Check sheet for the modelled part. Datum: model origin and axes. Units: mm. A direction names the side the tool comes from. Coordinates: 2 decimals unless noted, no trailing zeros. Loops run counter-clockwise (first coordinate to the right, second up) from the corner with the lowest first, then second, coordinate; pieces in that order, holes last. Notation, with made-up numbers: (-10, 5) - (38, 5) arc R29 cw to (38, 35) - close; hole circle Ø2 at (25.5, 74). An arc over 180 degrees is marked (long way). Use a Markdown table: item, result. Add a question column.
1) Tool access check on faces 1 (the flat face through (-7.922, 11, 7)), 2 (the flat face through (-22.41, -3.21, 14.51)), 3 (the flat face through (23, 1.722, 7)). Record the directions out of +Z, -Z, +X, -X, +Y, -Y that give a thin tool (end or side, any length) a straight path to the whole face; none if there is none.
2) Sectioned sample at A-A, the plane z = 7.5. Enter the section's corners in (x, y).
3) Sectioned sample at B-B, the plane y = -4.5. Enter the section's corners in (x, z).
4) Draft check along X on faces 4 (the flat face through (2, -8.278, 7)), 5 (the flat face through (27.078, -3, 7)), 6 (the cylindrical face through (16.53, -3.35, 8.76)). Enter one of: pulls with the +X half, pulls with the -X half, needs draft (parallel to the pull), parting line crosses it, or undercut.
5) Go/stop test with flat-tipped pins: P1, Ø1.5, axis at y = 4, z = 12, coming from the +X side; P2, Ø1, axis at x = -6, y = 12, coming from the -Z side; P3, Ø4, axis at x = 19.58, z = 7.5, coming from the +Y side; P4, Ø7.5, axis at x = -15.42, z = 7.5, coming from the +Y side. Record where each tip stops, or that it passes through.
6) Thickness scan on line 1 (X direction, y = 16.5, z = 11); line 2 (Y direction, x = -19, z = 2.5); line 3 (X direction, y = 14, z = 10). Record the ranges inside material, lowest first.
7) Sectioned sample at C-C, the plane y = 10. Enter the section's corners in (x, z), then the cut area to 3 significant figures.
8) Sectioned sample at D-D, the plane x = 22. Enter the section's corners in (y, z), then the cut area to 3 significant figures.
from build123d import *

# Parameters (mm, degrees)
BOSS_EXTRUDE1_DEPTH     = 15
CHAMFER1_SIZE           = 1
HOLE1_D                 = 6.6
M10X1_25_TAPPED_HOLE1_D = 8.8


with BuildPart() as part:
    # Sketch1 → Boss-Extrude1 (new body)
    with BuildSketch(Plane.XY):
        Polygon((-7.92160415, 21.721938776), (-7.92160415, 1.721938776), (-22.92160415, 1.721938776), (-22.92160415, -8.278061224), (27.07839585, -8.278061224), (27.07839585, 1.721938776), (12.07839585, 1.721938776), (12.07839585, 21.721938776), align=None)
    extrude(amount=BOSS_EXTRUDE1_DEPTH)

    # Chamfer1
    chamfer1_edges = [part.edges().sort_by_distance(p)[0] for p in [
        (-22.92160415, -3.278061224, 0),
        (12.07839585, 21.721938776, 7.5),
        (-7.92160415, 21.721938776, 7.5),
        (-22.92160415, -3.278061224, 15),
        (27.07839585, -3.278061224, 15),
        (27.07839585, -3.278061224, 0),
    ]]
    chamfer(chamfer1_edges, length=CHAMFER1_SIZE)

    # Hole1 (through all)
    with Locations(Plane(origin=(0, 1.721938776, 0), x_dir=(1, 0, 0), z_dir=(0, 1, 0))):
        with Locations((-15.42160415, -7.5), (19.57839585, -7.5)):
            Hole(HOLE1_D / 2)

    # M10x1.25 Tapped Hole1 (through all)
    with Locations(Plane.XY.offset(15)):
        with Locations((2.07839585, 10.721938776)):
            Hole(M10X1_25_TAPPED_HOLE1_D / 2)


solid = part.part
Solved:
| question | item | result |
|---|---|---|
| 1 | face 1 | +Z, -Z, -X, +Y |
| 1 | face 2 | +Z, -X, +Y, -Y |
| 1 | face 3 | +Z, -Z, +X, +Y |
| 2 | outline | (-22.92, -8.28) - (-18.72, -8.28) - (-18.72, 1.72) - (-22.92, 1.72) - close; (-12.12, -8.28) - (16.28, -8.28) - (16.28, 1.72) - (12.08, 1.72) - (12.08, 20.72) - (11.08, 21.72) - (-6.92, 21.72) - (-7.92, 20.72) - (-7.92, 1.72) - (-12.12, 1.72) - close; (22.88, -8.28) - (27.08, -8.28) - (27.08, 1.72) - (22.88, 1.72) - close; hole circle Ø8.8 at (2.08, 10.72) |
| 3 | outline | (-22.92, 1) - (-21.92, 0) - (26.08, 0) - (27.08, 1) - (27.08, 14) - (26.08, 15) - (-21.92, 15) - (-22.92, 14) - close; hole circle Ø6.6 at (-15.42, 7.5); hole circle Ø6.6 at (19.58, 7.5) |
| 4 | face 4 | needs draft |
| 4 | face 5 | pulls with the +X half |
| 4 | face 6 | undercut |
| 5 | P1 | stops at x = 12.08 |
| 5 | P2 | stops at z = 0 |
| 5 | P3 | passes through |
| 5 | P4 | stops at y = 1.72 |
| 6 | line 1 | x = -7.92 to 12.08 |
| 6 | line 2 | y = -8.28 to 1.72 |
| 6 | line 3 | x = -7.92 to -0.86, 5.01 to 12.08 |
| 7 | outline | (-7.92, 0) - (-2.26, 0) - (-2.26, 15) - (-7.92, 15) - close; (6.42, 0) - (12.08, 0) - (12.08, 15) - (6.42, 15) - close |
| 7 | area | 170 mm2 |
| 8 | outline | (-8.28, 0) - (1.72, 0) - (1.72, 5.26) - (-8.28, 5.26) - close; (-8.28, 9.74) - (1.72, 9.74) - (1.72, 15) - (-8.28, 15) - close |
| 8 | area | 105 mm2 |
